The listing builds one solid part. Answer for the finished solid, in the listing's coordinates (mm). A direction names the side the tool comes from. Coordinates: 2 decimals unless noted, no trailing zeros. Order: outer loops, then holes, each group sorted by start corner. A loop starts at its lowest first (then second) coordinate and runs counter-clockwise, first axis right, second up. Notation, with made-up numbers: (43.5, 45.25) - (57.5, 45.25) arc R26 ccw to (57.5, 84.25) - close; hole circle Ø11 at (70, 36.5). An arc over 180 degrees is marked (long way). Use a Markdown table: item, result. Add a question column.
Item 1: The part is cut by section B-B, the plane z = 24. Give the vertices of the cut face in (x, y).
Item 2: The part is cut by section A-A, the plane z = 65. Give the vertices of the cut face in (x, y).
Item 3: Find the intervals of material crossed by line 1 along Z through (x, y) = (0, 5); line 2 along Z through (x, y) = (7, 6.85); line 3 along X through (y, z) = (3, 24), in increasing order.
Item 4: Flat-ended cylindrical pins translate along their axes: P1, Ø5, axis at x = -7, z = 24, coming from the -Y side; P2, Ø3.5, axis at x = -7, z = -24, coming from the +Y side. Find the tip coordinate at first contact, or state that the pin passes through.
Item 5: The mould has two halves that part along X. Classify faces 1 (the flat face through (12, 4, 1)), 2 (the flat face through (5, 4.4, 26)), 3 (the flat face through (0, 4, 85)): released by +X, released by -X, zero draft, split by the parting line, or undercut.
Item 6: The part is cut by section C-C, the plane y = 2.75. State how many separate pieces and enclosed holes the cut face has, then the cut area to 3 significant figures.
Item 7: For faces 4 (the cylindrical face through (1.666, 3.944, 81.278)), 5 (the cylindrical face through (-6.479, 2.169, 20.034)), determine the directions among +Z, -Z, +X, -X, +Y, -Y from which every point of the face is accessible in a straight line to the end or side of a thin tool.
Item 8: The part is cut by section D-D, the plane x = -7. Give the vertices of the cut face in (y, z).
from build123d import *

# Parameters (mm, degrees)
SKETCH_1_W                   = 24
SKETCH_1_H                   = 170
EXTRUDE_1_DEPTH              = 8
HOLE_WIZARD_M4_1_D           = 4.5
HOLE_WIZARD_M4_1_CBORE_D     = 8
HOLE_WIZARD_M4_1_CBORE_DEPTH = 4.4
HOLE_WIZARD_M5_1_D           = 4.2
HOLE_WIZARD_M5_1_DEPTH       = 12.4
HOLE_WIZARD_M5_1_TIP         = 1.2618073
CHAMFER_1_SIZE               = 2
CHAMFER_2_SIZE               = 0.5


with BuildPart() as part:
    # 草图1 → 凸台-拉伸1 (new body)
    with BuildSketch(Plane(origin=(0, 0, 0), x_dir=(1, 0, 0), z_dir=(0, 1, 0))):
        Rectangle(SKETCH_1_W, SKETCH_1_H)
    extrude(amount=EXTRUDE_1_DEPTH)

    # M4 六角凹头螺钉的柱形沉头孔1 (through all)
    with Locations(Plane(origin=(0, 0, 0), x_dir=(-1, 0, 0), z_dir=(0, -1, 0))):
        with Locations((-7, 24), (7, 24), (-7, -24), (7, -24)):
            CounterBoreHole(HOLE_WIZARD_M4_1_D / 2, HOLE_WIZARD_M4_1_CBORE_D / 2, HOLE_WIZARD_M4_1_CBORE_DEPTH)

    # M5 螺纹孔1
    with Locations(Plane(origin=(0, 8, 0), x_dir=(1, 0, 0), z_dir=(0, 1, 0))):
        with Locations((0, 80), (0, -80), (0, -65), (0, 65)):
            Hole(HOLE_WIZARD_M5_1_D / 2, depth=HOLE_WIZARD_M5_1_DEPTH)
            with Locations((0, 0, -(HOLE_WIZARD_M5_1_DEPTH + HOLE_WIZARD_M5_1_TIP / 2))):  # 118° drill point
                Cone(0, HOLE_WIZARD_M5_1_D / 2, HOLE_WIZARD_M5_1_TIP, mode=Mode.SUBTRACT)

    # 倒角1
    chamfer_1_edges = [part.edges().sort_by_distance(p)[0] for p in [
        (12, 4, 85),
        (-12, 4, 85),
        (-12, 4, -85),
        (12, 4, -85),
    ]]
    chamfer(chamfer_1_edges, length=CHAMFER_1_SIZE)

    # 倒角2
    chamfer_2_edges = [part.edges().sort_by_distance(p)[0] for p in [
        (-12, 0, 0),
        (-12, 8, 0),
        (12, 0, 0),
        (0, 0, 85),
        (0, 0, -85),
        (11, 0, 84),
        (-11, 0, 84),
        (11, 0, -84),
        (-11, 0, -84),
        (0, 8, -85),
        (12, 8, 0),
        (0, 8, 85),
        (11, 8, 84),
        (-11, 8, 84),
        (11, 8, -84),
        (-11, 8, -84),
    ]]
    chamfer(chamfer_2_edges, length=CHAMFER_2_SIZE)


solid = part.part
Solution:
| question | item | result |
|---|---|---|
| 1 | outline | (-12, 0.5) - (-11.5, 0) - (-11, 0) - (-11, 4.4) - (-9.25, 4.4) - (-9.25, 8) - (-11.5, 8) - (-12, 7.5) - close; (-4.75, 4.4) - (-3, 4.4) - (-3, 0) - (3, 0) - (3, 4.4) - (4.75, 4.4) - (4.75, 8) - (-4.75, 8) - close; (9.25, 4.4) - (11, 4.4) - (11, 0) - (11.5, 0) - (12, 0.5) - (12, 7.5) - (11.5, 8) - (9.25, 8) - close |
| 2 | outline | (-12, 0.5) - (-11.5, 0) - (-2.1, 0) - (-2.1, 8) - (-11.5, 8) - (-12, 7.5) - close; (2.1, 0) - (11.5, 0) - (12, 0.5) - (12, 7.5) - (11.5, 8) - (2.1, 8) - close |
| 3 | line 1 | z = -85 to -82.1, -77.9 to -67.1, -62.9 to 62.9, 67.1 to 77.9, 82.1 to 85 |
| 3 | line 2 | z = -85 to -26.25, -21.75 to 21.75, 26.25 to 85 |
| 3 | line 3 | x = -12 to -11, -3 to 3, 11 to 12 |
| 4 | P1 | stops at y = 4.4 |
| 4 | P2 | passes through |
| 5 | face 1 | released by +X |
| 5 | face 2 | undercut |
| 5 | face 3 | zero draft |
| 6 | separate pieces | 1 |
| 6 | enclosed holes | 8 |
| 6 | area | 3,820 mm2 |
| 7 | face 4 | +Y, -Y |
| 7 | face 5 | -Y |
| 8 | outline | (0, -84.5) - (0.5, -85) - (7.5, -85) - (8, -84.5) - (8, -26.25) - (4.4, -26.25) - (4.4, -28) - (0, -28) - close; (0, -20) - (4.4, -20) - (4.4, -21.75) - (8, -21.75) - (8, 21.75) - (4.4, 21.75) - (4.4, 20) - (0, 20) - close; (0, 28) - (4.4, 28) - (4.4, 26.25) - (8, 26.25) - (8, 84.5) - (7.5, 85) - (0.5, 85) - (0, 84.5) - close |
